Check sheet for the modelled part. Datum: model origin and axes. Units: mm. Face numbers are marked on the shaded views. Give positions to 0.01 mm unless a question says otherwise; leave off trailing zeros. Order: outer loops, then holes, each group sorted by start corner. A loop starts at its lowest first (then second) coordinate and runs counter-clockwise, first axis right, second up. Notation, with made-up numbers: (12, 20.5) - (28, 20.5) arc R25 cw to (28, 44.5) - close; hole circle Ø2 at (74, 5.5). An arc over 180 degrees is marked (long way). Answer in a Markdown table with one row per item.
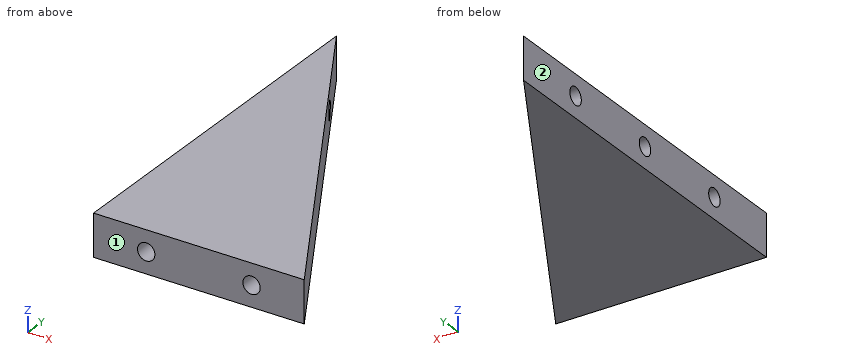
from build123d import *

# Parameters (mm, degrees)
EXTRUDE_1_DEPTH        = 8
HOLE_WIZARD_M4_1_D     = 3.3
HOLE_WIZARD_M4_1_DEPTH = 12
HOLE_WIZARD_M4_1_TIP   = 0.991420021
HOLE_WIZARD_M4_2_D     = 3.3
HOLE_WIZARD_M4_2_DEPTH = 12
HOLE_WIZARD_M4_2_TIP   = 0.991420021


with BuildPart() as part:
    # 草图1 → 凸台-拉伸1 (new body)
    with BuildSketch(Plane.XY):
        Polygon((-20, -35), (20, -35), (-20, 35), align=None)
    extrude(amount=EXTRUDE_1_DEPTH)

    # M4 螺纹孔1
    with Locations(Plane.ZY.offset(20)):
        with Locations((4, -20), (4, 0), (4, 20)):
            Hole(HOLE_WIZARD_M4_1_D / 2, depth=HOLE_WIZARD_M4_1_DEPTH)
            with Locations((0, 0, -(HOLE_WIZARD_M4_1_DEPTH + HOLE_WIZARD_M4_1_TIP / 2))):  # 118° drill point
                Cone(0, HOLE_WIZARD_M4_1_D / 2, HOLE_WIZARD_M4_1_TIP, mode=Mode.SUBTRACT)

    # M4 螺纹孔2
    with Locations(Plane(origin=(0, -35, 0), x_dir=(-1, 0, 0), z_dir=(0, -1, 0))):
        with Locations((-10, -4), (10, -4)):
            Hole(HOLE_WIZARD_M4_2_D / 2, depth=HOLE_WIZARD_M4_2_DEPTH)
            with Locations((0, 0, -(HOLE_WIZARD_M4_2_DEPTH + HOLE_WIZARD_M4_2_TIP / 2))):  # 118° drill point
                Cone(0, HOLE_WIZARD_M4_2_D / 2, HOLE_WIZARD_M4_2_TIP, mode=Mode.SUBTRACT)


solid = part.part
(1) Cross-section at C-C, the plane y = -26. Record the cut outline in (x, z), then the cut area to 3 significant figures.
Geometry says:
| item | result |
|---|---|
| outline | (-20, 0) - (14.86, 0) - (14.86, 8) - (-20, 8) - close; hole circle Ø3.3 at (-10, 4); hole circle Ø3.3 at (10, 4) |
| area | 262 mm² |
(2) Gauge pin test, flat ends, axial feed: P1, Ø3, axis at y = 20, z = 4, coming from the -X side; P2, Ø3, axis at x = 10, z = 4, coming from the -Y side; P3, Ø4, axis at x = -10, z = 4, coming from the +Y side. Record the tip position at first contact, or that the pin passes through.
Geometry says:
| item | result |
|---|---|
| P1 | through |
| P2 | y = -22.91 |
| P3 | y = 19.6 |
(3) Mould release check, pull along X, two halves, no side actions. Record for the marked faces 1 and 2: pulls with the +X half, pulls with the -X half, needs draft (parallel to the pull), parting line crosses it, or undercut.
Geometry says:
| item | result |
|---|---|
| face 1 | needs draft |
| face 2 | pulls with the -X half |
(4) Cross-section at A-A, the plane y = 20. Record the cut outline in (x, z), then the cut area to 3 significant figures.
Geometry says:
| item | result |
|---|---|
| outline | (-20, 0) - (-11.43, 0) - (-11.43, 2.35) - (-20, 2.35) - close; (-20, 5.65) - (-11.43, 5.65) - (-11.43, 8) - (-20, 8) - close |
| area | 40.3 mm² |
(5) Thickness scan on L1, parallel to Z at x = 10, y = -28; L2, parallel to X at y = -28, z = 3; L3, parallel to Y at x = -17.75, z = 4. Record the ranges inside material, lowest first.
Geometry says:
| item | result |
|---|---|
| L1 | 0 to 2.35, 5.65 to 8 |
| L2 | -20 to -11.31, -8.69 to 8.69, 11.31 to 16 |
| L3 | -35 to -21.65, -18.35 to -1.65, 1.65 to 18.35, 21.65 to 31.06 |
(6) Cross-section at B-B, the plane z = 1. Record the cut outline in (x, y), then the cut area to 3 significant figures.
Geometry says:
| item | result |
|---|---|
| outline | (-20, -35) - (20, -35) - (-20, 35) - close |
| area | 1,400 mm² |
(7) Cross-section at D-D, the plane x = 5.5. Record the cut outline in (y, z) (3 decimals).
Geometry says:
| item | result |
|---|---|
| outline | (-35, 0) - (-9.625, 0) - (-9.625, 8) - (-35, 8) - close |
